For this review, take the finished solid that the model builds, in its own axes (mm). Give positions to 0.01 mm unless a question says otherwise; leave off trailing zeros. Write each loop counter-clockwise with the first axis right and the second up, starting at its lowest first coordinate (ties: lowest second). Pieces come first, ordered by that corner, then holes. Notation, with made-up numbers: M 24.25,-8.75 L 76.25,-8.75 A12 ccw 76.25,7.25 Z; hole C -1,44 d7. An arc over 180 degrees is marked long. Use one line per item in the form item = value. Start each with the question number.
Q1. For probe 1 along Y at (x, z) = (112, 14.25); probe 2 along Y at (x, z) = (440, 17.5); probe 3 along Y at (x, z) = (413, 19), list the stretches that pass through material, from the lowest coordinate up. Write a range as [from, to].
Q2. Clearance check with flat-ended pins moving along their axes: pin 1 Ø4 at (x, z) = (315.5, 20) entering from -Y; pin 2 Ø1 at (y, z) = (271.5, 18) entering from +X. State where each tip first meets the part, or that it passes through.
Q3. Consider section D-D on y = 193. Write out the cut boundary in (x, z), and give its area (3 significant figures).
Q4. Consider section C-C on x = 149.5. Write out the cut boundary in (y, z).
Q5. Consider section B-B on z = 17.75. Write out the cut boundary in (x, y), and give its area (3 significant figures).
Q6. Consider section A-A on y = 369.5. Write out the cut boundary in (x, z), and give its area (3 significant figures).
```python
from build123d import *

# Parameters (mm, degrees)
SKETCH1_R           = 42.5
BOSS_EXTRUDE1_DEPTH = 30


with BuildPart() as part:
    # Sketch1 → Boss-Extrude1 (new body)
    with BuildSketch(Plane.XY):
        with BuildLine():
            Line((0, 0), (0, 420))
            Line((0, 420), (300, 420))
            Line((300, 420), (300, 460))
            Line((300, 460), (413, 460))
            ThreePointArc((413, 460), (491.066504669, 415.280682048), (491.982051466, 325.317587819))
            Line((491.982051466, 325.317587819), (310, 0))
            Line((310, 0), (0, 0))
        make_face()
        with Locations((413, 369.5)):
            Circle(SKETCH1_R, mode=Mode.SUBTRACT)
    extrude(amount=BOSS_EXTRUDE1_DEPTH)


solid = part.part
```
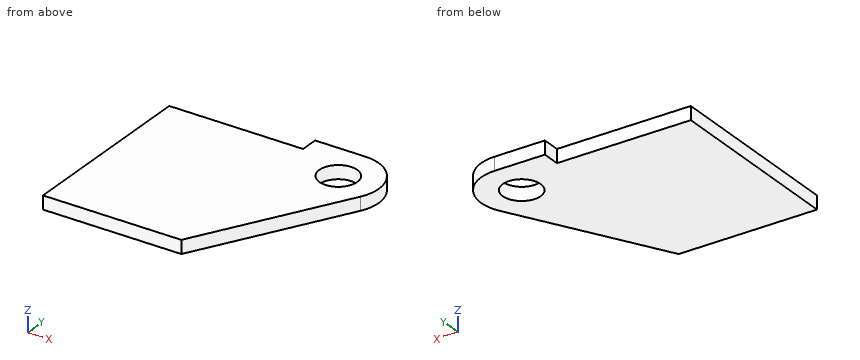
Working result:
q1.probe_1 = [0, 420]
q1.probe_2 = [232.39, 336.68], [402.32, 455.88]
q1.probe_3 = [184.13, 327], [412, 460]
q2.pin_1 = 6.26
q2.pin_2 = 462.16
q3.outline = M 0,0 L 417.96,0 L 417.96,30 L 0,30 Z
q3.area = 12,500 mm²
q4.outline = M 0,0 L 420,0 L 420,30 L 0,30 Z
q5.outline = M 0,0 L 310,0 L 491.98,325.32 A90.5 ccw 413,460 L 300,460 L 300,420 L 0,420 Z; hole C 413,369.5 d85
q5.area = 179,000 mm²
q6.outline = M 0,0 L 370.5,0 L 370.5,30 L 0,30 Z; M 455.5,0 L 503.5,0 L 503.5,30 L 455.5,30 Z
q6.area = 12,600 mm²
